Build history of the part. All positions in model axes, mm. A direction names the side the tool comes from. Round coordinates to 2 decimals unless told otherwise and drop trailing zeros. Write each loop counter-clockwise with the first axis right and the second up, starting at its lowest first coordinate (ties: lowest second). Pieces come first, ordered by that corner, then holes. Notation, with made-up numbers: (37.5, 36.25) - (50.5, 36.25) arc R19 cw to (50.5, 70.25) - close; hole circle Ø6 at (-4, 80.25). An arc over 180 degrees is marked (long way). Answer as a JSON object with one key per item and string values. Group by question number.
Item 1: Slice it at C-C, the plane y = 0. List the corners of the cut face in (x, z), then the cut area to 3 significant figures.
Item 2: Flat gauge pins, fed straight in: pin 1 (6 mm diameter, centred on y = -0.5, z = 36.5, fed in from +X); pin 2 (5 mm diameter, centred on x = 6, z = 7.5, fed in from +Y); pin 3 (5 mm diameter, centred on x = 4, y = 1.5, fed in from -Z); pin 4 (5 mm diameter, centred on x = -1, y = -1, fed in from +Z). Where does each tip first touch, or does it go through?
Item 3: Slice it at A-A, the plane z = 53. List the corners of the cut face in (x, y).
Item 4: Slice it at D-D, the plane z = 35. List the corners of the cut face in (x, y).
Item 5: Two-plate mould, pull along X, no slides. Class faces 1 (the flat face through (5.2, 0.1, 60)), 2 (the flat face through (4.984, 0.405, 56.056)), 3 (the cylindrical face through (-1.73, -7.81, 54.93)): +X half, -X half, draft (parallel to the pull), parting line (faces both ways), or undercut.
Item 6: Which spindle directions (+Z, -Z, +X, -X, +Y, -Y) get a long thin tool onto all of the face, cutting with end or side? Do faces 4 (the flat face through (5.2, 0.1, 50)), 5 (the flat face through (0, 0, 0)), 6 (the flat face through (-4.984, -0.405, 56.056)). Say none if no direction does.
Item 7: Slice it at B-B, the plane x = -2.5. List the corners of the cut face in (y, z).
Item 8: Probe line 1 (Z direction, x = -4.5, y = -3.5); line 2 (Z direction, x = -4, y = -2.75); line 3 (Y direction, x = 0.25, z = 42). List the from-to ranges inside material, lowest first. Write a range as from..to.
from build123d import *

# Parameters (mm, degrees)
SKETCH1_R           = 5
BOSS_EXTRUDE1_DEPTH = 50
SKETCH2_R           = 8
BOSS_EXTRUDE2_DEPTH = 10
CUT_EXTRUDE1_DEPTH  = 8


with BuildPart() as part:
    # Sketch1 → Boss-Extrude1 (new body)
    with BuildSketch(Plane.XY):
        Circle(SKETCH1_R)
    extrude(amount=BOSS_EXTRUDE1_DEPTH)

    # Sketch2 → Boss-Extrude2 (add)
    with BuildSketch(Plane.XY.offset(50)):
        Circle(SKETCH2_R)
    extrude(amount=BOSS_EXTRUDE2_DEPTH)

    # Sketch3 → Cut-Extrude1 (cut)
    with BuildSketch(Plane.XY.offset(60)):
        Polygon((0.514138009, -5.750564793), (5.237204202, -2.430025819), (4.723066192, 3.320538974), (-0.514138009, 5.750564793), (-5.237204202, 2.430025819), (-4.723066192, -3.320538974), align=None)
    extrude(amount=-CUT_EXTRUDE1_DEPTH, mode=Mode.SUBTRACT)


solid = part.part
Geometry says:
{
 "1": {"outline": "(-8, 50) - (-5, 50) - (-5, 0) - (5, 0) - (5, 50) - (8, 50) - (8, 60) - (5.02, 60) - (5.02, 52) - (-5.02, 52) - (-5.02, 60) - (-8, 60) - close", "area": "580 mm^2"},
 "2": {"pin 1": "stops at x = 5", "pin 2": "stops at y = 3.57", "pin 3": "stops at z = 0", "pin 4": "stops at z = 52"},
 "3": {"outline": "circle Ø16 at (0, 0); hole (-5.24, 2.43) - (-4.72, -3.32) - (0.51, -5.75) - (5.24, -2.43) - (4.72, 3.32) - (-0.51, 5.75) - close"},
 "4": {"outline": "circle Ø10 at (0, 0)"},
 "5": {"face 1": "draft", "face 2": "undercut", "face 3": "parting line"},
 "6": {"face 4": "-Z", "face 5": "-Z, +X, -X, +Y, -Y", "face 6": "+Z"},
 "7": {"outline": "(-7.6, 50) - (-4.33, 50) - (-4.33, 0) - (4.33, 0) - (4.33, 50) - (7.6, 50) - (7.6, 60) - (4.35, 60) - (4.35, 52) - (-4.35, 52) - (-4.35, 60) - (-7.6, 60) - close"},
 "8": {"line 1": "z = 50..60", "line 2": "z = 0..52", "line 3": "y = -4.99..4.99"}
}
